Verification items for the finished model (mm, model axes). A direction names the side the tool comes from. Coordinates: 2 decimals unless noted, no trailing zeros. Answer as CSV lines item,"result". Start each with the question number.
1. Material ranges on line 1 (Y direction, x = -139, z = -3); line 2 (X direction, y = 17.5, z = 0.5); line 3 (Y direction, x = -147, z = 3.75), recorded low to high. Write a range as [from, to].
2. Set-up check for faces 1 (the flat face through (250, -22, 0)), 2 (the flat face through (304, -36, 0)), 3 (the flat face through (-35, -3, 0.2)): record each of +Z, -Z, +X, -X, +Y, -Y from which the full face is reachable in a straight line by a thin tool's end or side.
3. Release check for a two-part mould opening along X. For faces 4 (the flat face through (61, -29, 0.2)), 5 (the flat face through (-3, 50, 0)), 6 (the flat face through (199, 13, 0)), 7 (the cylindrical face through (55.505, -2.758, 3.648)) record: pulls with the +X half, pulls with the -X half, needs draft (parallel to the pull), parting line crosses it, or undercut.
4. Gauge pin test, flat ends, axial feed: P1, Ø5.5, axis at x = 59, y = -24, coming from the +Z side; P2, Ø4, axis at y = 26, z = 5, coming from the +X side; P3, Ø4, axis at x = -89, z = 0, coming from the -Y side. Record the tip position at first contact, or that the pin passes through.
```python
from build123d import *

# Parameters (mm, degrees)
SKETCH1_W                                            = 398
SKETCH1_H                                            = 100
BOSS_EXTRUDE1_DEPTH                                  = 7
SKETCH2_W                                            = 14
SKETCH2_H                                            = 28
BOSS_EXTRUDE2_DEPTH                                  = 105
M6_CLEARANCE_HOLE1_D                                 = 6.6
M6_TAPPED_HOLE1_D                                    = 5
HOLE_SIZE_PER_SOCKET_HEAD_CAP_SCREW_TYPE_D           = 6.6
HOLE_SIZE_PER_SOCKET_HEAD_CAP_SCREW_TYPE_CBORE_D     = 11
HOLE_SIZE_PER_SOCKET_HEAD_CAP_SCREW_TYPE_CBORE_DEPTH = 6.8
M6_TAPPED_HOLE2_D                                    = 5
M6_TAPPED_HOLE3_D                                    = 5
M6_TAPPED_HOLE3_DEPTH                                = 15
M6_TAPPED_HOLE3_TIP                                  = 1.502151548
CHAMFER1_SIZE                                        = 1


with BuildPart() as part:
    # Sketch1 → Boss-Extrude1 (new, symmetric)
    with BuildSketch(Plane.XY):
        Rectangle(SKETCH1_W, SKETCH1_H)
    extrude(amount=BOSS_EXTRUDE1_DEPTH, both=True)

    # Sketch2 → Boss-Extrude2 (add)
    with BuildSketch(Plane(origin=(199, 0, 0), x_dir=(0, 0, -1), z_dir=(1, 0, 0))):
        with Locations((0, -36)):
            Rectangle(SKETCH2_W, SKETCH2_H)
    extrude(amount=BOSS_EXTRUDE2_DEPTH)

    # M6 Clearance Hole1 (through all)
    with Locations(Plane(origin=(0, 0, -7), x_dir=(-1, 0, 0), z_dir=(0, 0, -1))):
        with Locations((-254, -43), (-254, -29)):
            Hole(M6_CLEARANCE_HOLE1_D / 2)

    # M6 Tapped Hole1 (through all)
    with Locations(Plane.XY.offset(7)):
        with Locations((111, -13), (-189, 33), (-189, -13), (-89, 33), (-89, -13), (11, 33), (11, -13), (111, 33)):
            Hole(M6_TAPPED_HOLE1_D / 2)

    # Hole Size per Socket Head Cap Screw Type1 (through all)
    with Locations(Plane.XY.offset(7)):
        with Locations((-139, -3), (61, -25), (61, -3), (-39, -25), (-39, -3), (-139, -25)):
            CounterBoreHole(HOLE_SIZE_PER_SOCKET_HEAD_CAP_SCREW_TYPE_D / 2, HOLE_SIZE_PER_SOCKET_HEAD_CAP_SCREW_TYPE_CBORE_D / 2, HOLE_SIZE_PER_SOCKET_HEAD_CAP_SCREW_TYPE_CBORE_DEPTH)

    # M6 Tapped Hole2 (through all)
    with Locations(Plane(origin=(0, 0, -7), x_dir=(-1, 0, 0), z_dir=(0, 0, -1))):
        with Locations((-191, 43), (-147, 17), (-191, 17), (-147, 43), (147, 43), (191, 17), (147, 17), (191, 43)):
            Hole(M6_TAPPED_HOLE2_D / 2)

    # M6 Tapped Hole3
    with Locations(Plane(origin=(0, -50, 0), x_dir=(-1, 0, 0), z_dir=(0, -1, 0))):
        with Locations((-291, 0), (189, 0), (89, 0), (-11, 0), (-111, 0), (-211, 0)):
            Hole(M6_TAPPED_HOLE3_D / 2, depth=M6_TAPPED_HOLE3_DEPTH)
            with Locations((0, 0, -(M6_TAPPED_HOLE3_DEPTH + M6_TAPPED_HOLE3_TIP / 2))):  # 118° drill point
                Cone(0, M6_TAPPED_HOLE3_D / 2, M6_TAPPED_HOLE3_TIP, mode=Mode.SUBTRACT)

    # Chamfer1
    chamfer1_edges = [part.edges().sort_by_distance(p)[0] for p in [
        (304, -50, 0),
        (304, -22, 0),
        (-199, -50, 0),
        (-199, 50, 0),
        (199, 50, 0),
    ]]
    chamfer(chamfer1_edges, length=CHAMFER1_SIZE)


solid = part.part
```
Values follow:
1,line 1,"y = [-50, -28.3], [-21.7, -6.3], [0.3, 50]"
1,line 2,"x = [-199, -193.45], [-188.55, -149.45], [-144.55, 144.55], [149.45, 188.55], [193.45, 199]"
1,line 3,"y = [-50, 14.5], [19.5, 40.5], [45.5, 50]"
2,face 1,"+Z, -Z, +X, +Y"
2,face 2,"+Z, -Z, +X, +Y, -Y"
2,face 3,"+Z"
3,face 4,"undercut"
3,face 5,"needs draft"
3,face 6,"pulls with the +X half"
3,face 7,"undercut"
4,P1,"stops at z = 0.2"
4,P2,"stops at x = 199"
4,P3,"stops at y = -34.7"
